Part model, mm, in its own coordinate system. A direction names the side the tool comes from. Round coordinates to 2 decimals unless told otherwise and drop trailing zeros. Loops run counter-clockwise (first coordinate to the right, second up) from the corner with the lowest first, then second, coordinate; pieces in that order, holes last.
(1) Mould opens along X. For faces 1 (the face through (10, 28, 4)), 2 (the face through (-18, 3, 4)), 3 (the face through (0, 37, 8)) say: +X half, -X half, draft (parallel to the pull), parting line (faces both ways), or undercut.
(2) Tool access for faces 4 (the face through (6, 15, 4)), 5 (the face through (18, 3, 4)): list every direction of +Z, -Z, +X, -X, +Y, -Y with a clear straight run to the whole face (end or side of a thin tool).
(3) Flat gauge pin, fed straight in: pin 1 (8 mm diameter, centred on x = -7.5, y = 15, fed in from -Z). Where does the tip first touch, or does it go through?
(4) Cut at D-D on y = 54. List the corners of the cut face in (x, z).
(5) Cut at A-A on y = 20. List the corners of the cut face in (x, z).
(6) Probe probe 1 along X at (y, z) = (14, 6.75); probe 2 along Y at (x, z) = (-2.5, 1.5); probe 3 along Y at (x, z) = (-3.5, 1.5). List the from-to ranges inside material, lowest first.
(7) Cut at B-B on z = 6. List the corners of the cut face in (x, y).
(8) Cut at C-C on x = -3. List the corners of the cut face in (y, z).
from build123d import *

# Parameters (mm, degrees)
EXTRUDE_1_DEPTH = 8
CHAMFER_1_SIZE  = 5


with BuildPart() as part:
    # 草图1 → 凸台-拉伸1 (new body)
    # profile 1 of 2: a face of its own
    with BuildSketch(Plane.XY):
        with BuildLine():
            Line((-20, 45), (-20, 0))
            Line((-20, 0), (0, 0))
            Line((0, 0), (0, 52))
            ThreePointArc((0, 52), (-5, 57), (0, 62))
            Line((0, 62), (0, 72))
            Line((0, 72), (-10.64516129, 72))
            Line((-10.64516129, 72), (-20, 45))
        make_face()
        with BuildLine():
            ThreePointArc((-6, 7), (-10, 3), (-14, 7))
            Line((-14, 7), (-14, 24))
            ThreePointArc((-14, 24), (-10, 28), (-6, 24))
            Line((-6, 24), (-6, 7))
        make_face(mode=Mode.SUBTRACT)
    # profile 2 of 2: a face of its own
    with BuildSketch(Plane.XY):
        with BuildLine():
            Line((0, 52), (0, 0))
            Line((0, 0), (20, 0))
            Line((20, 0), (20, 45))
            Line((20, 45), (10.64516129, 72))
            Line((10.64516129, 72), (0, 72))
            Line((0, 72), (0, 62))
            ThreePointArc((0, 62), (3.535533906, 60.535533906), (5, 57))
            ThreePointArc((5, 57), (3.535533906, 53.464466094), (0, 52))
        make_face()
        with BuildLine():
            ThreePointArc((14, 7), (10, 3), (6, 7))
            Line((6, 7), (6, 24))
            ThreePointArc((6, 24), (10, 28), (14, 24))
            Line((14, 24), (14, 7))
        make_face(mode=Mode.SUBTRACT)
    extrude(amount=EXTRUDE_1_DEPTH)

    # 倒角1
    chamfer_1_edges = [part.edges().sort_by_distance(p)[0] for p in [
        (-20, 0, 4),
        (20, 0, 4),
    ]]
    chamfer(chamfer_1_edges, length=CHAMFER_1_SIZE)


solid = part.part
Final values:
1. face 1: undercut
1. face 2: -X half
1. face 3: draft
2. face 4: +Z, -Z
2. face 5: +Z, -Z, +X, -Y
3. pin 1: stops at z = 0
4. outline: (-16.88, 0) - (-4, 0) - (-4, 8) - (-16.88, 8) - close; (4, 0) - (16.88, 0) - (16.88, 8) - (4, 8) - close
5. outline: (-20, 0) - (-14, 0) - (-14, 8) - (-20, 8) - close; (-6, 0) - (6, 0) - (6, 8) - (-6, 8) - close; (14, 0) - (20, 0) - (20, 8) - (14, 8) - close
6. probe 1: x = -20 to -14, -6 to 6, 14 to 20
6. probe 2: y = 0 to 52.67, 61.33 to 72
6. probe 3: y = 0 to 53.43, 60.57 to 72
7. outline: (-20, 5) - (-15, 0) - (15, 0) - (20, 5) - (20, 45) - (10.65, 72) - (-10.65, 72) - (-20, 45) - close; hole (-14, 7) arc R4 ccw to (-6, 7) - (-6, 24) arc R4 ccw to (-14, 24) - close; hole circle Ø10 at (0, 57); hole (6, 7) arc R4 ccw to (14, 7) - (14, 24) arc R4 ccw to (6, 24) - close
8. outline: (0, 0) - (53, 0) - (53, 8) - (0, 8) - close; (61, 0) - (72, 0) - (72, 8) - (61, 8) - close
